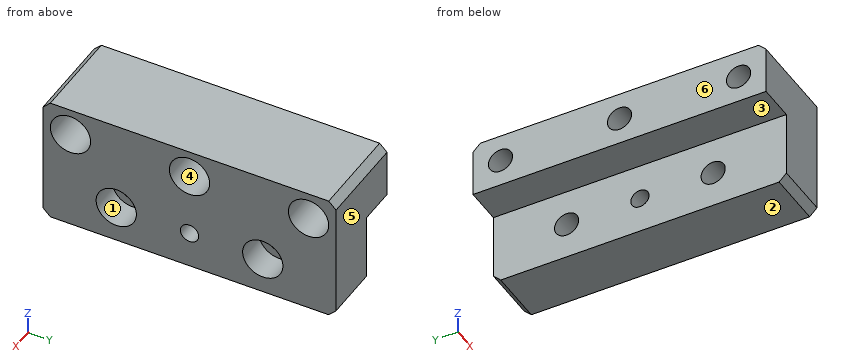
from build123d import *

# Parameters (mm, degrees)
EXTRUDE_1_DEPTH              = 40
CHAMFER_1_SIZE               = 2
HOLE_WIZARD_M6_1_D           = 6.6
HOLE_WIZARD_M6_1_CBORE_D     = 11
HOLE_WIZARD_M6_1_CBORE_DEPTH = 15
HOLE_WIZARD_M6_1_2_D         = 5
HOLE_WIZARD_M6_2_D           = 6.6
HOLE_WIZARD_M6_2_CBORE_D     = 11
HOLE_WIZARD_M6_2_CBORE_DEPTH = 8


with BuildPart() as part:
    # 草图1 → 凸台-拉伸1 (new, symmetric)
    with BuildSketch(Plane(origin=(0, 0, 0), x_dir=(1, 0, 0), z_dir=(0, 1, 0))):
        Polygon((0, 0), (25, 0), (25, 35), (10, 35), (10, 15), (0, 15), align=None)
    extrude(amount=EXTRUDE_1_DEPTH, both=True)

    # 倒角1
    chamfer_1_edges = [part.edges().sort_by_distance(p)[0] for p in [
        (17.5, 40, -35),
        (17.5, -40, -35),
        (12.5, -40, 0),
        (12.5, 40, 0),
    ]]
    chamfer(chamfer_1_edges, length=CHAMFER_1_SIZE)

    # Hole Wizard M6 _1 (through all)
    with Locations(Plane(origin=(25, 0, 0), x_dir=(0, 0, -1), z_dir=(1, 0, 0))):
        with Locations((7.5, 32.5), (7.5, 0), (7.5, -32.5)):
            CounterBoreHole(HOLE_WIZARD_M6_1_D / 2, HOLE_WIZARD_M6_1_CBORE_D / 2, HOLE_WIZARD_M6_1_CBORE_DEPTH)

    # Hole Wizard M6 _1 2 (through all)
    with Locations(Plane(origin=(25, 0, 0), x_dir=(0, 0, -1), z_dir=(1, 0, 0))):
        with Locations((25, 0)):
            Hole(HOLE_WIZARD_M6_1_2_D / 2)

    # M6 六角圆柱头螺钉的柱形沉头孔2 (through all)
    with Locations(Plane(origin=(25, 0, 0), x_dir=(0, 0, -1), z_dir=(1, 0, 0))):
        with Locations((25, 20), (25, -20)):
            CounterBoreHole(HOLE_WIZARD_M6_2_D / 2, HOLE_WIZARD_M6_2_CBORE_D / 2, HOLE_WIZARD_M6_2_CBORE_DEPTH)


solid = part.part
Check sheet for the modelled part. Datum: model origin and axes. Units: mm. Face numbers are marked on the shaded views. A direction names the side the tool comes from. Give positions to 0.01 mm unless a question says otherwise; leave off trailing zeros. Loops run counter-clockwise (first coordinate to the right, second up) from the corner with the lowest first, then second, coordinate; pieces in that order, holes last. Notation, with made-up numbers: M 38.25,64.25 L 90.25,64.25 A9 ccw 90.25,79.25 Z; hole C 12,51 d4. An arc over 180 degrees is marked long. Answer as a JSON object with one key per item and string values. Group by question number.
Q1. Release check for a two-part mould opening along Y. For the marked faces 4, 5 and 6 record: released by +Y, released by -Y, zero draft, split by the parting line, or undercut.
Q2. Cross-section at D-D on z = -7.5. Record the cut outline in (x, y).
Q3. Material ranges on line 1 along Y through (x, z) = (4, -7.5); line 2 along Y through (x, z) = (13.5, -25); line 3 along Z through (x, y) = (5.5, -10), recorded low to high. Write a range as [from, to].
Q4. Go/stop test with flat-tipped pins: P1, Ø6.5, axis at y = -32.5, z = -7.5, coming from the -X side; P2, Ø10.5, axis at y = -20, z = -25, coming from the +X side; P3, Ø10, axis at y = 32.5, z = -7.5, coming from the +X side; P4, Ø5, axis at y = 25.5, z = -25.5, coming from the -X side. Record where each tip stops, or that it passes through.
Q5. Access from +Z, -Z, +X, -X, +Y, -Y to the whole of each face (thin tool, end or side, straight path). Record for the marked faces 1, 2 and 3.
Q6. Cross-section at B-B on x = 8. Record the cut outline in (y, z), then the cut area to 3 significant figures.
Q7. Cross-section at A-A on y = 32.5. Record the cut outline in (x, z), then the cut area to 3 significant figures.
Q8. Cross-section at C-C on y = 0. Record the cut outline in (x, z), then the cut area to 3 significant figures.
Evaluation:
{
 "1": {"face 4": "undercut", "face 5": "released by +Y", "face 6": "zero draft"},
 "2": {"outline": "M 0,-40 L 25,-40 L 25,-38 L 10,-38 L 10,-35.8 L 0,-35.8 Z; M 0,-29.2 L 10,-29.2 L 10,-27 L 25,-27 L 25,-5.5 L 10,-5.5 L 10,-3.3 L 0,-3.3 Z; M 0,3.3 L 10,3.3 L 10,5.5 L 25,5.5 L 25,27 L 10,27 L 10,29.2 L 0,29.2 Z; M 0,35.8 L 10,35.8 L 10,38 L 25,38 L 25,40 L 0,40 Z"},
 "3": {"line 1": "y = [-40, -35.8], [-29.2, -3.3], [3.3, 29.2], [35.8, 40]", "line 2": "y = [-40, -23.3], [-16.7, -2.5], [2.5, 16.7], [23.3, 40]", "line 3": "z = [-15, 0]"},
 "4": {"P1": "passes through", "P2": "stops at x = 17", "P3": "stops at x = 10", "P4": "stops at x = 10"},
 "5": {"face 1": "+X", "face 2": "-Z, +X, -X, +Y, -Y", "face 3": "-Z, -X, +Y, -Y"},
 "6": {"outline": "M -40,-15 L 40,-15 L 40,-2 L 38,0 L -38,0 L -40,-2 Z; hole C -32.5,-7.5 d6.6; hole C 0,-7.5 d6.6; hole C 32.5,-7.5 d6.6", "area": "1,090 mm2"},
 "7": {"outline": "M 0,-15 L 10,-15 L 10,-35 L 25,-35 L 25,-13 L 10,-13 L 10,-10.8 L 0,-10.8 Z; M 0,-4.2 L 10,-4.2 L 10,-2 L 25,-2 L 25,0 L 0,0 Z", "area": "444 mm2"},
 "8": {"outline": "M 0,-15 L 10,-15 L 10,-22.5 L 25,-22.5 L 25,-13 L 10,-13 L 10,-10.8 L 0,-10.8 Z; M 0,-4.2 L 10,-4.2 L 10,-2 L 25,-2 L 25,0 L 0,0 Z; M 10,-35 L 25,-35 L 25,-27.5 L 10,-27.5 Z", "area": "369 mm2"}
}
